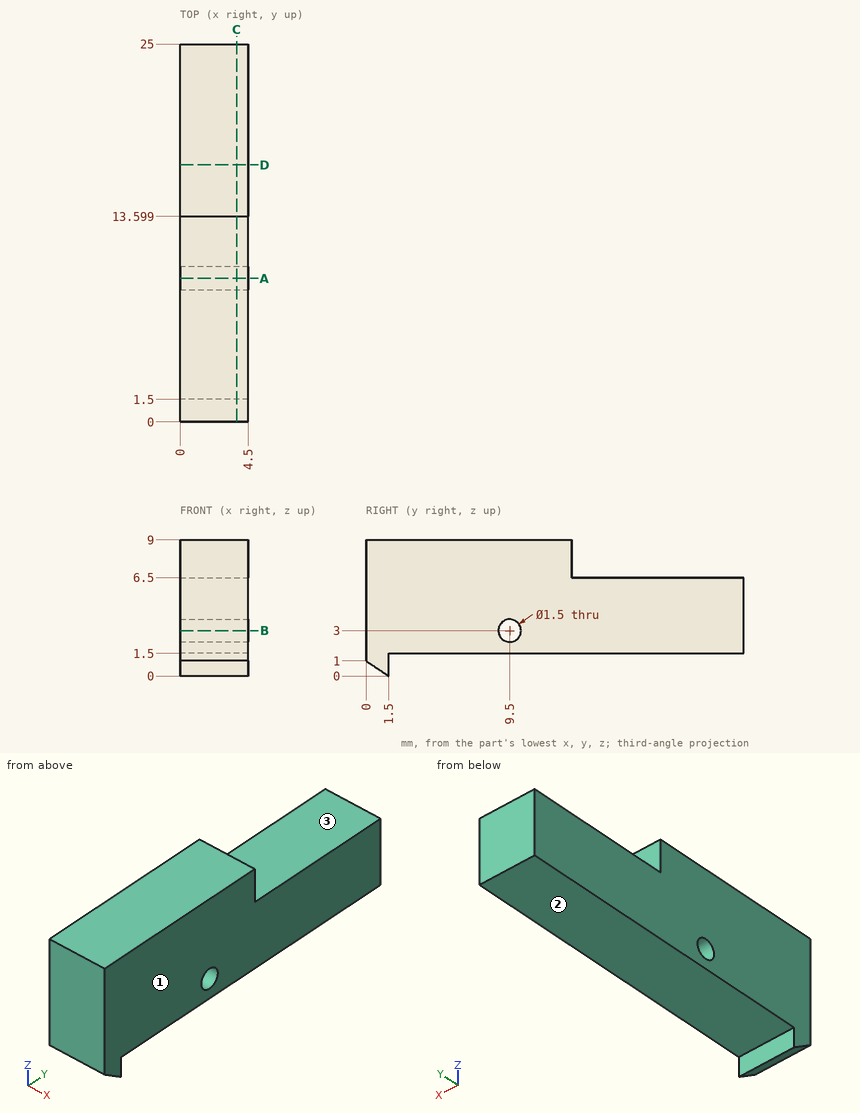
The figure shows three views and two pictorial views of one solid part (mm, origin at its lowest corner). Answer the questions. A direction names the side the tool comes from. Give positions to 0.01 mm unless a question says otherwise; leave off trailing zeros. Write each loop counter-clockwise with the first axis right and the second up, starting at its lowest first coordinate (ties: lowest second). Pieces come first, ordered by that corner, then holes. Notation, with made-up numbers: (61.5, 76) - (116.5, 76) arc R26 cw to (116.5, 105) - close; hole circle Ø4 at (-22.75, 55). An arc over 180 degrees is marked (long way). Use one line per item in the form item = value.
1. A cutting plane is placed at C-C (x = 3.75). Write down the section's boundary in (y, z), and give its area (3 significant figures).
Filled in:
outline = (0, 1) - (1.5, 0) - (1.5, 1.5) - (25, 1.5) - (25, 6.5) - (13.6, 6.5) - (13.6, 9) - (0, 9) - close; hole circle Ø1.5 at (9.5, 3)
area = 159 mm^2
2. A cutting plane is placed at B-B (z = 3). Write down the section's boundary in (x, y).
Filled in:
outline = (0, 0) - (4.5, 0) - (4.5, 8.75) - (0, 8.75) - close; (0, 10.25) - (4.5, 10.25) - (4.5, 25) - (0, 25) - close
3. Each of these flat-tipped pins is pushed along its axis until it touches: pin 1 Ø2 at (x, y) = (2.5, 21.5) entering from +Z; pin 2 Ø2 at (x, z) = (2.5, 8) entering from +Y; pin 3 Ø1.5 at (x, y) = (3.5, 15) entering from -Z. Where does it stop, or does it pass through?
Filled in:
pin_1 = 6.5
pin_2 = 13.6
pin_3 = 1.5
4. A cutting plane is placed at D-D (y = 17). Write down the section's boundary in (x, z).
Filled in:
outline = (0, 1.5) - (4.5, 1.5) - (4.5, 6.5) - (0, 6.5) - close
5. A cutting plane is placed at A-A (y = 9.5). Write down the section's boundary in (x, z), and give its area (3 significant figures).
Filled in:
outline = (0, 1.5) - (4.5, 1.5) - (4.5, 2.25) - (0, 2.25) - close; (0, 3.75) - (4.5, 3.75) - (4.5, 9) - (0, 9) - close
area = 27.0 mm^2
6. Consider L1, parallel to Z at x = 3.05, y = 9.5; L2, parallel to Z at x = 3.6, y = 3; L3, parallel to Z at x = 2.25, y = 14.75. Determine where each line is inside the solid, lowest interval first.
Filled in:
L1 = 1.5 to 2.25, 3.75 to 9
L2 = 1.5 to 9
L3 = 1.5 to 6.5
7. For the marked faces 1, 2 and 3, determine the directions among +Z, -Z, +X, -X, +Y, -Y from which every point of the face is accessible in a straight line to the end or side of a thin tool.
Filled in:
face_1 = +Z, -Z, +X, +Y, -Y
face_2 = -Z, +X, -X, +Y
face_3 = +Z, +X, -X, +Y
